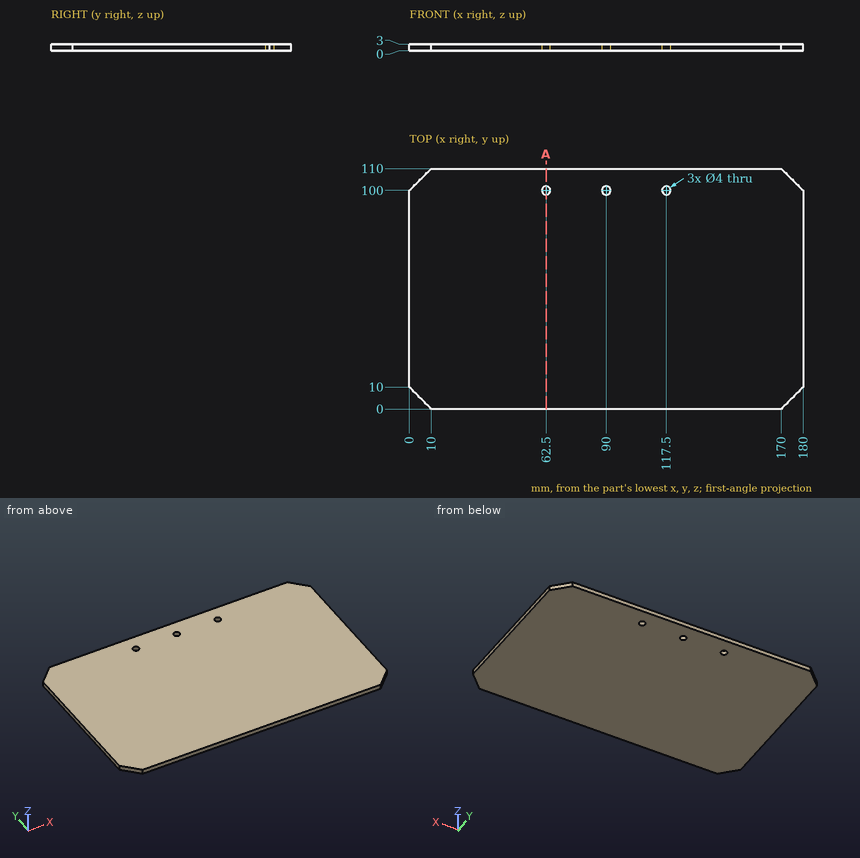
For this review, use the dimensioned drawing (mm, ordinates from the lowest corner) and the shaded views. Round coordinates to 2 decimals unless told otherwise and drop trailing zeros. Loops run counter-clockwise (first coordinate to the right, second up) from the corner with the lowest first, then second, coordinate; pieces in that order, holes last. Notation, with made-up numbers: M 3,29 L 53,29 A24 ccw 53,57 Z; hole C 15.25,74 d3. An arc over 180 degrees is marked long. Answer as CSV lines item,"result".
1. To check wall thickness, follow L1, parallel to Y at x = 117.5, z = 1.8; L2, parallel to X at y = 7, z = 2.15; L3, parallel to X at y = 106, z = 1.25. State the ranges of each line that lie inside material, in increasing order. Write a range as [from, to].
Outcome:
L1,"y = [0, 98], [102, 110]"
L2,"x = [3, 177]"
L3,"x = [6, 174]"
2. We need section A-A (x = 62.5). Give the boundary of the cut face in (y, z).
Outcome:
outline,"M 0,0 L 98,0 L 98,3 L 0,3 Z; M 102,0 L 110,0 L 110,3 L 102,3 Z"
3. Insertion check: pin 1 Ø2.5 at (x, y) = (62.5, 100) entering from -Z. The pin has a flat end and moves straight along its axis. Give the tip position at first contact, or say it passes through.
Outcome:
pin 1,"passes through"
